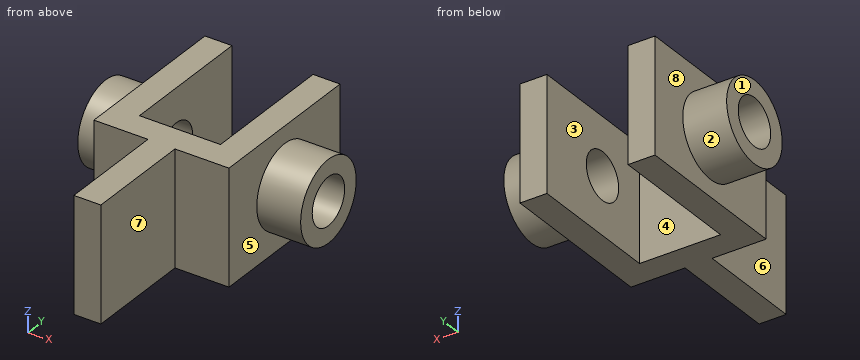
from build123d import *

# Parameters (mm, degrees)
FORK_BODY_DEPTH          = 34
SIDE_BOSS_A_SKETCH_R     = 12
SIDE_BOSS_A_SKETCH_R_2   = 7
SIDE_BOSS_A_24X_14_DEPTH = 13
SIDE_START               = 13
SIDE_BOSS_B_SKETCH_R     = 12
SIDE_BOSS_B_SKETCH_R_2   = 7
SIDE_BOSS_B_24X_14_DEPTH = 13
PIN_HOLE_SKETCH_R        = 7
PIN_HOLE_DEPTH           = 102.808644034


with BuildPart() as part:
    # Fork Profile Sketch → Fork Body (new body)
    with BuildSketch(Plane.XY):
        Polygon((-2.871912694, 0), (-2.871912694, 32), (-18.871912694, 32), (-18.871912694, 80), (-10.871912694, 80), (-10.871912694, 40), (13.128087306, 40), (13.128087306, 80), (21.128087306, 80), (21.128087306, 32), (5.128087306, 32), (5.128087306, 0), align=None)
    extrude(amount=-FORK_BODY_DEPTH)

    # Side Boss A Sketch → Side Boss A Ø24xØ14 (add)
    with BuildSketch(Plane(origin=(21.128087306, 0, 0), x_dir=(0, 0, -1), z_dir=(1, 0, 0))):
        with Locations(Location((17, 56, 0), (0, 0, 270))):
            Circle(SIDE_BOSS_A_SKETCH_R)
        with Locations(Location((17, 56, 0), (0, 0, 270))):
            Circle(SIDE_BOSS_A_SKETCH_R_2, mode=Mode.SUBTRACT)
    extrude(amount=SIDE_BOSS_A_24X_14_DEPTH)

    # Side Boss B Sketch → Side Boss B Ø24xØ14 (add)
    with BuildSketch(Plane.ZY.offset(18.871912694).offset(SIDE_START)):
        with Locations(Location((-17, 56, 0), (0, 0, 270))):
            Circle(SIDE_BOSS_B_SKETCH_R)
        with Locations(Location((-17, 56, 0), (0, 0, 270))):
            Circle(SIDE_BOSS_B_SKETCH_R_2, mode=Mode.SUBTRACT)
    extrude(amount=-SIDE_BOSS_B_24X_14_DEPTH)

    # Pin Hole Sketch → Pin Hole (cut, through all)
    with BuildSketch(Plane.ZY.offset(18.871912694)):
        with Locations(Location((-17, 56, 0), (0, 0, 270))):
            Circle(PIN_HOLE_SKETCH_R)
    extrude(amount=-PIN_HOLE_DEPTH, mode=Mode.SUBTRACT)


solid = part.part
CAD build for the part. Positions are in the model's coordinates, mm. Face numbers are marked on the shaded views. A direction names the side the tool comes from. Coordinates: 2 decimals unless noted, no trailing zeros. Write each loop counter-clockwise with the first axis right and the second up, starting at its lowest first coordinate (ties: lowest second). Pieces come first, ordered by that corner, then holes. Notation, with made-up numbers: M -36,-27 L 11,-27 A20 cw 11,2 Z; hole C -37.75,53 d3. An arc over 180 degrees is marked long. Answer as a JSON object with one key per item and string values. Group by question number.
1) Saw through at D-D (x = 24). Write the cut outline in (y, z).
2) Saw through at C-C (y = 56). Write the cut outline in (x, z), plus the area to 3 significant figures.
3) Mould opens along X. For the marked faces 1, 2 and 3 say: +X half, -X half, draft (parallel to the pull), parting line (faces both ways), or undercut.
4) Tool access for the marked faces 4, 5, 6, 7 and 8: list every direction of +Z, -Z, +X, -X, +Y, -Y with a clear straight run to the whole face (end or side of a thin tool).
5) Wall check: line 1 (X direction, y = 65, z = -13); line 2 (X direction, y = 46, z = -29); line 3 (Z direction, x = -20, y = 56). Give the ranges that are in metal, low to high. Write a range as from..to.
6) Saw through at B-B (z = -17). Write the cut outline in (x, y).
7) Pin check, flat tips, straight feed: pin 1 Ø3 at (y, z) = (16, -17.5) entering from -X; pin 2 Ø6 at (y, z) = (14, -13) entering from +X; pin 3 Ø11 at (y, z) = (56, -17) entering from +X; pin 4 Ø10 at (x, z) = (-21, -7) entering from -Y. Stop position of each tip, or through.
8) Saw through at A-A (y = 73). Write the cut outline in (x, z).
Values follow:
{
 "1": {"outline": "C 56,-17 d24; hole C 56,-17 d14"},
 "2": {"outline": "M -31.87,-29 L -18.87,-29 L -18.87,-34 L -10.87,-34 L -10.87,-24 L -31.87,-24 Z; M -31.87,-10 L -10.87,-10 L -10.87,0 L -18.87,0 L -18.87,-5 L -31.87,-5 Z; M 13.13,-34 L 21.13,-34 L 21.13,-29 L 34.13,-29 L 34.13,-24 L 13.13,-24 Z; M 13.13,-10 L 34.13,-10 L 34.13,-5 L 21.13,-5 L 21.13,0 L 13.13,0 Z", "area": "580 mm2"},
 "3": {"face 1": "-X half", "face 2": "draft", "face 3": "undercut"},
 "4": {"face 4": "+Z, -Z, +Y", "face 5": "+X", "face 6": "+Z, -Z, -X, -Y", "face 7": "+Z, -Z, +X, -Y", "face 8": "-X"},
 "5": {"line 1": "x = -31.87..-10.87, 13.13..34.13", "line 2": "x = -18.87..-10.87, 13.13..21.13", "line 3": "z = -29..-24, -10..-5"},
 "6": {"outline": "M -31.87,44 L -18.87,44 L -18.87,32 L -2.87,32 L -2.87,0 L 5.13,0 L 5.13,32 L 21.13,32 L 21.13,44 L 34.13,44 L 34.13,49 L 13.13,49 L 13.13,40 L -10.87,40 L -10.87,49 L -31.87,49 Z; M -31.87,63 L -10.87,63 L -10.87,80 L -18.87,80 L -18.87,68 L -31.87,68 Z; M 13.13,63 L 34.13,63 L 34.13,68 L 21.13,68 L 21.13,80 L 13.13,80 Z"},
 "7": {"pin 1": "stops at x = -2.87", "pin 2": "stops at x = 5.13", "pin 3": "passes through", "pin 4": "stops at y = 32"},
 "8": {"outline": "M -18.87,-34 L -10.87,-34 L -10.87,0 L -18.87,0 Z; M 13.13,-34 L 21.13,-34 L 21.13,0 L 13.13,0 Z"}
}
